Read the model definition and answer for the solid it produces. Units are mm, in the model's axes. Round coordinates to 2 decimals unless told otherwise and drop trailing zeros. Order: outer loops, then holes, each group sorted by start corner. A loop starts at its lowest first (then second) coordinate and runs counter-clockwise, first axis right, second up. Notation, with made-up numbers: M 0.25,84 L 10.25,84 A18 cw 10.25,112 Z; hole C 58.5,42 d4. An arc over 180 degrees is marked long. Use one line per item in the form item = value. Start each with the question number.
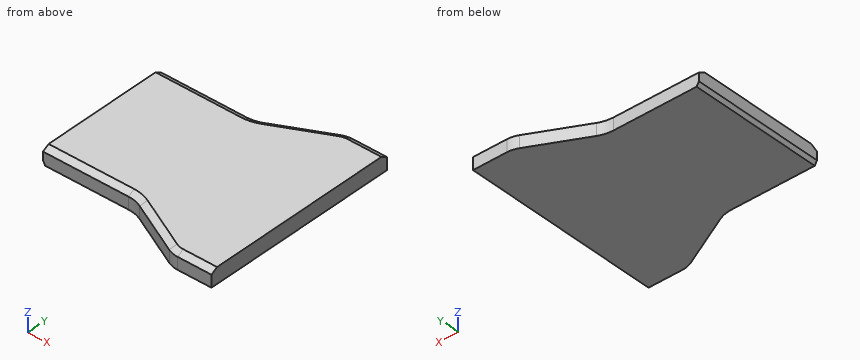
from build123d import *

# Parameters (mm, degrees)
EXTRUDE_1_DEPTH = 20
CHAMFER_1_SIZE  = 8
CHAMFER_1_SIZE2 = 4.618802154
CHAMFER_3_SIZE  = 5
CHAMFER_3_SIZE2 = 2.886751346


with BuildPart() as part:
    # 草图1 → 凸台-拉伸1 (new body)
    with BuildSketch(Plane.XY):
        with BuildLine():
            Line((-305.507868128, -251), (-322.917960675, -251))
            ThreePointArc((-322.917960675, -251), (-329.810548291, -250.197469684), (-336.33436854, -247.83281573))
            Line((-336.33436854, -247.83281573), (-403.66563146, -214.16718427))
            ThreePointArc((-403.66563146, -214.16718427), (-412.364058458, -211.014312331), (-421.55417528, -209.94427191))
            Line((-421.55417528, -209.94427191), (-530, -209.94427191))
            Line((-530, -209.94427191), (-530, -41.05572809))
            Line((-530, -41.05572809), (-421.55417528, -41.05572809))
            ThreePointArc((-421.55417528, -41.05572809), (-412.364058458, -39.985687669), (-403.66563146, -36.83281573))
            Line((-403.66563146, -36.83281573), (-336.33436854, -3.16718427))
            ThreePointArc((-336.33436854, -3.16718427), (-329.810548291, -0.802530316), (-322.917960675, 0))
            Line((-322.917960675, 0), (-300, 0))
            Line((-300, 0), (-280, 0))
            Line((-280, 0), (-280, -251))
            Line((-280, -251), (-305.507868128, -251))
        make_face()
    extrude(amount=-EXTRUDE_1_DEPTH)

    # 倒角1
    chamfer_1_edges = [part.edges().sort_by_distance(p)[0] for p in [
        (-301.458980338, -251, 0),
        (-329.810548291, -250.197469684, 0),
        (-370, -231, 0),
        (-412.364058458, -211.014312331, 0),
        (-475.77708764, -209.94427191, 0),
        (-475.77708764, -41.05572809, 0),
        (-412.364058458, -39.985687669, 0),
        (-370, -20, 0),
        (-329.810548291, -0.802530316, 0),
        (-301.458980338, 0, 0),
    ]]
    chamfer_1_side = [part.faces().sort_by_distance(p)[0] for p in [
        (-393.523242802, -125.5, 0),
    ]]
    chamfer(chamfer_1_edges, length=CHAMFER_1_SIZE, length2=CHAMFER_1_SIZE2, reference=chamfer_1_side[0])

    # 倒角3
    chamfer_3_edges = [part.edges().sort_by_distance(p)[0] for p in [
        (-530, -125.5, -20),
    ]]
    chamfer_3_side = [part.faces().sort_by_distance(p)[0] for p in [
        (-530, -125.5, -10.093574404),
    ]]
    chamfer(chamfer_3_edges, length=CHAMFER_3_SIZE, length2=CHAMFER_3_SIZE2, reference=chamfer_3_side[0])


solid = part.part
Item 1: Given P1, Ø3, axis at x = -343, z = -4.5, coming from the +Y side; P2, Ø4, axis at x = -457.5, z = -3.5, coming from the -Y side; P3, Ø2, axis at x = -499, z = -9.5, coming from the +Y side, each flat-ended and moving along its own axis, determine where each tip first touches the part or whether it passes through.
Item 2: Section A-A (z = -10.75) is taken. Write down the section's boundary in (x, y), and give its area (3 significant figures).
Item 3: Section D-D (x = -455) is taken. Write down the section's boundary in (y, z).
Item 4: Section B-B (x = -396) is taken. Write down the section's boundary in (y, z), and give its area (3 significant figures).
Item 5: Section C-C (y = -28) is taken. Write down the section's boundary in (x, z).
Item 6: Find the intervals of material crossed by L1, parallel to Y at x = -483, z = -5; L2, parallel to Y at x = -420, z = -10.75; L3, parallel to X at y = -26.5, z = -4.75, in increasing order. Write a range as [from, to].
The answers:
q1.P1 = -5.75
q1.P2 = -209.94
q1.P3 = -41.06
q2.outline = M -530,-209.94 L -421.55,-209.94 A40 cw -403.67,-214.17 L -336.33,-247.83 A30 ccw -322.92,-251 L -280,-251 L -280,0 L -322.92,0 A30 ccw -336.33,-3.17 L -403.67,-36.83 A40 cw -421.55,-41.06 L -530,-41.06 Z
q2.area = 49,700 mm²
q3.outline = M -209.94,-20 L -41.06,-20 L -41.06,-4.62 L -49.06,0 L -201.94,0 L -209.94,-4.62 Z
q4.outline = M -218,-20 L -33,-20 L -33,-4.62 L -41.94,0 L -209.06,0 L -218,-4.62 Z
q4.area = 3,660 mm²
q5.outline = M -386,-20 L -280,-20 L -280,0 L -368.11,0 L -386,-4.62 Z
q6.L1 = [-209.94, -41.06]
q6.L2 = [-209.97, -41.03]
q6.L3 = [-383, -280]
